CAD build for the part. Positions are in the model's coordinates, mm. Face numbers are marked on the shaded views. A direction names the side the tool comes from. Round coordinates to 2 decimals unless told otherwise and drop trailing zeros. Order: outer loops, then holes, each group sorted by start corner. A loop starts at its lowest first (then second) coordinate and runs counter-clockwise, first axis right, second up. Notation, with made-up numbers: M 17.5,16 L 25.5,16 A31 cw 25.5,40 Z; hole C 21.25,64.5 d10. An arc over 180 degrees is marked long. Answer as CSV lines item,"result". Start each with the question number.
```python
from build123d import *

# Parameters (mm, degrees)
SKETCH1_R           = 3
BOSS_EXTRUDE1_DEPTH = 6
SKETCH2_R           = 10
BOSS_EXTRUDE2_DEPTH = 13
FILLET1_R           = 2


with BuildPart() as part:
    # Sketch1 → Boss-Extrude1 (new body)
    with BuildSketch(Plane(origin=(0, 0, 0), x_dir=(1, 0, 0), z_dir=(0, 1, 0))):
        with BuildLine():
            Line((-24, 13), (24, 13))
            ThreePointArc((24, 13), (37, 0), (24, -13))
            Line((24, -13), (-24, -13))
            ThreePointArc((-24, -13), (-37, 0), (-24, 13))
        make_face()
        with Locations(Location((-24, 0, 0), (0, 0, 270))):
            Circle(SKETCH1_R, mode=Mode.SUBTRACT)
        with Locations(Location((24, 0, 0), (0, 0, 270))):
            Circle(SKETCH1_R, mode=Mode.SUBTRACT)
    extrude(amount=BOSS_EXTRUDE1_DEPTH)

    # Sketch2 → Boss-Extrude2 (add, symmetric)
    with BuildSketch(Plane.XY):
        with BuildLine():
            Line((-14, 20), (-14, 0))
            Line((-14, 0), (14, 0))
            Line((14, 0), (14, 20))
            ThreePointArc((14, 20), (0, 34), (-14, 20))
        make_face()
        with Locations(Location((0, 20, 0), (0, 0, 180))):
            Circle(SKETCH2_R, mode=Mode.SUBTRACT)
    extrude(amount=BOSS_EXTRUDE2_DEPTH, both=True)

    # Fillet1
    fillet1_edges = [part.edges().sort_by_distance(p)[0] for p in [
        (-14, 6, 0),
        (14, 6, 0),
    ]]
    fillet(fillet1_edges, radius=FILLET1_R)


solid = part.part
```
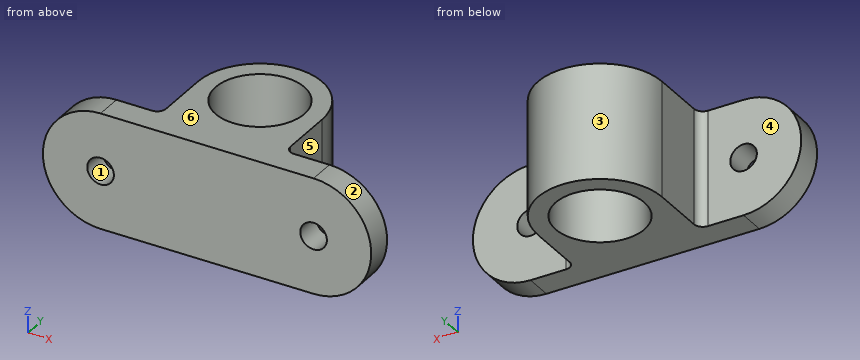
Q1. Band-saw the part on C-C, the plane y = 26.5. Write the cut outline in (x, z), then the cut area to 3 significant figures.
Q2. Band-saw the part on A-A, the plane x = 0. Write the cut outline in (y, z).
Q3. Tool access for the marked faces 4, 5 and 6: list every direction of +Z, -Z, +X, -X, +Y, -Y with a clear straight run to the whole face (end or side of a thin tool).
Q4. Mould opens along X. For the marked faces 1, 2 and 3 say: +X half, -X half, draft (parallel to the pull), parting line (faces both ways), or undercut.
Q5. Band-saw the part on D-D, the plane z = 11. Write the cut outline in (x, y).
Q6. Band-saw the part on B-B, the plane z = 1.75. Write the cut outline in (x, y).
Q7. Drop flat-ended pins along their axis: P1, Ø13, axis at y = 13, z = -1, coming from the -X side; P2, Ø10.5, axis at x = -26, z = -5, coming from the +Y side; P3, Ø5, axis at y = 3.5, z = 4.5, coming from the +X side; P4, Ø10, axis at x = 5.5, z = -10, coming from the -Y side. Give the stop position or say it passes through.
Q8. Probe line 1 along X through (y, z) = (20, 0); line 2 along Y through (x, z) = (7.5, 11); line 3 along Y through (x, z) = (3, 5). List the from-to ranges inside material, lowest first. Write a range as from..to.
Answer:
1,outline,"M -12.4,-13 L -7.6,-13 L -7.6,13 L -12.4,13 Z; M 7.6,-13 L 12.4,-13 L 12.4,13 L 7.6,13 Z"
1,area,"250 mm^2"
2,outline,"M 0,-13 L 10,-13 L 10,13 L 0,13 Z; M 30,-13 L 34,-13 L 34,13 L 30,13 Z"
3,face 4,"+Z, -Z, -X, +Y"
3,face 5,"+Z, -Z, +X, +Y"
3,face 6,"+Z, +X, -X, +Y, -Y"
4,face 1,"undercut"
4,face 2,"+X half"
4,face 3,"parting line"
5,outline,"M -30.93,0 L 30.93,0 L 30.93,6 L 16,6 A2 cw 14,8 L 14,20 A14 ccw -14,20 L -14,8 A2 cw -16,6 L -30.93,6 Z; hole C 0,20 d20"
6,outline,"M -36.88,0 L -26.44,0 L -26.44,6 L -36.88,6 Z; M -21.56,0 L 21.56,0 L 21.56,6 L 16,6 A2 cw 14,8 L 14,20 A14 ccw -14,20 L -14,8 A2 cw -16,6 L -21.56,6 Z; M 26.44,0 L 36.88,0 L 36.88,6 L 26.44,6 Z; hole C 0,20 d20"
7,P1,"stops at x = -14.68"
7,P2,"stops at y = 6"
7,P3,"stops at x = 36.85"
7,P4,"stops at y = 0"
8,line 1,"x = -14..-10, 10..14"
8,line 2,"y = 0..13.39, 26.61..31.82"
8,line 3,"y = 0..10.46, 29.54..33.67"
